For this review, use the dimensioned drawing (mm, ordinates from the lowest corner) and the shaded views. A direction names the side the tool comes from. Round coordinates to 2 decimals unless told otherwise and drop trailing zeros. Order: outer loops, then holes, each group sorted by start corner. A loop starts at its lowest first (then second) coordinate and runs counter-clockwise, first axis right, second up. Notation, with made-up numbers: (46.25, 56) - (80.25, 56) arc R22 ccw to (80.25, 63) - close; hole circle Ø11 at (18.5, -8.75). An arc over 180 degrees is marked (long way). Write item = value, one per line.
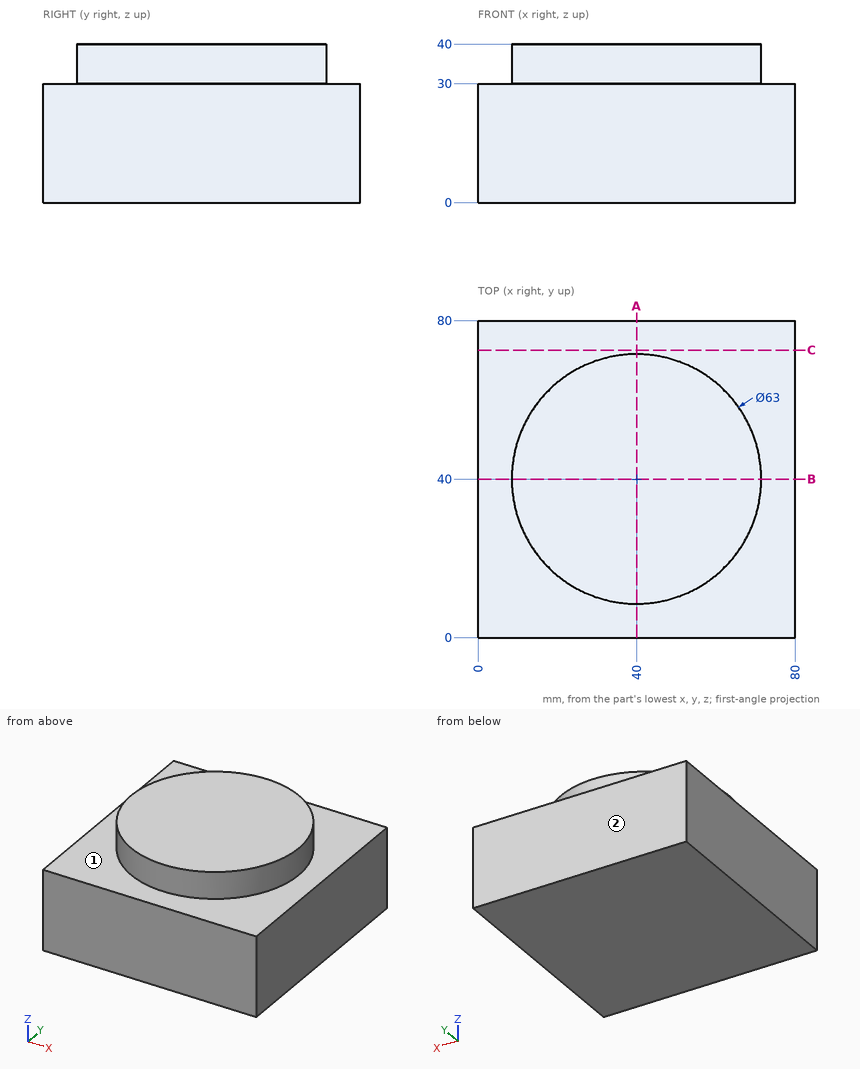
1) We need section C-C on y = 72.5. Write out the cut boundary in (x, z), and give its area (3 significant figures).
Findings:
outline = (0, 0) - (80, 0) - (80, 30) - (0, 30) - close
area = 2,400 mm^2
2) For the marked faces 1 and 2, list the 3-axis set-ups (+Z, -Z, +X, -X, +Y, -Y) from which the entire face can be reached by the end or side of a thin tool; tool diameter is ignored.
Findings:
face_1 = +Z
face_2 = +Z, -Z, +X, -X, +Y
3) We need section A-A on x = 40. Write out the cut boundary in (y, z), and give its area (3 significant figures).
Findings:
outline = (0, 0) - (80, 0) - (80, 30) - (71.5, 30) - (71.5, 40) - (8.5, 40) - (8.5, 30) - (0, 30) - close
area = 3,030 mm^2
4) To check wall thickness, follow L1, parallel to Z at x = 4, y = 16; L2, parallel to Y at x = 36, z = 33.5 (3 decimals); L3, parallel to X at y = 28.5, z = 34.5. State the ranges of each line that lie inside material, in increasing order. Write a range as from..to.
Findings:
L1 = 0..30
L2 = 8.755..71.245
L3 = 10.67..69.33
5) Clearance check with a flat-ended pin moving along its axis: pin 1 Ø2 at (x, y) = (58, 71) entering from +Z. State where the tip first meets the part, or that it passes through.
Findings:
pin_1 = 30
